```python
from build123d import *

# Parameters (mm, degrees)
EXTRUDE_1_DEPTH     = 7
FILLET_1_R          = 5
CUT_EXTRUDE_1_REACH = 193.047
SKETCH_3_R          = 3.5


with BuildPart() as part:
    # 草图1 → 凸台-拉伸1 (new, symmetric)
    with BuildSketch(Plane.XY):
        Polygon((0, 150), (-15, 150), (-15, 15), (-135, 15), (-135, 0), (0, 0), align=None)
    extrude(amount=EXTRUDE_1_DEPTH, both=True)

    # 圆角1
    fillet_1_edges = [part.edges().sort_by_distance(p)[0] for p in [
        (-15, 15, 0),
    ]]
    fillet(fillet_1_edges, radius=FILLET_1_R)

    # 草图3 → 切除-拉伸1 (cut, up to next)
    with BuildSketch(Plane(origin=(0, 15, 0), x_dir=(1, 0, 0), z_dir=(0, 1, 0)), mode=Mode.PRIVATE) as cut_extrude_1_sk1:
        with Locations(Location((-127, 0, 0), (0, 0, 180))):
            Circle(SKETCH_3_R)
    cut_extrude_1_tool1 = extrude(cut_extrude_1_sk1.sketch, amount=-CUT_EXTRUDE_1_REACH, mode=Mode.PRIVATE) & part.part
    # 草图3 → 切除-拉伸1 (cut, up to next)
    with BuildSketch(Plane(origin=(0, 15, 0), x_dir=(1, 0, 0), z_dir=(0, 1, 0)), mode=Mode.PRIVATE) as cut_extrude_1_sk2:
        with Locations(Location((-105, 0, 0), (0, 0, 180))):
            Circle(SKETCH_3_R)
    cut_extrude_1_tool2 = extrude(cut_extrude_1_sk2.sketch, amount=-CUT_EXTRUDE_1_REACH, mode=Mode.PRIVATE) & part.part
    add(cut_extrude_1_tool1.solids().sort_by_distance((-127, 15, 0))[0], mode=Mode.SUBTRACT)
    add(cut_extrude_1_tool2.solids().sort_by_distance((-105, 15, 0))[0], mode=Mode.SUBTRACT)


solid = part.part
```
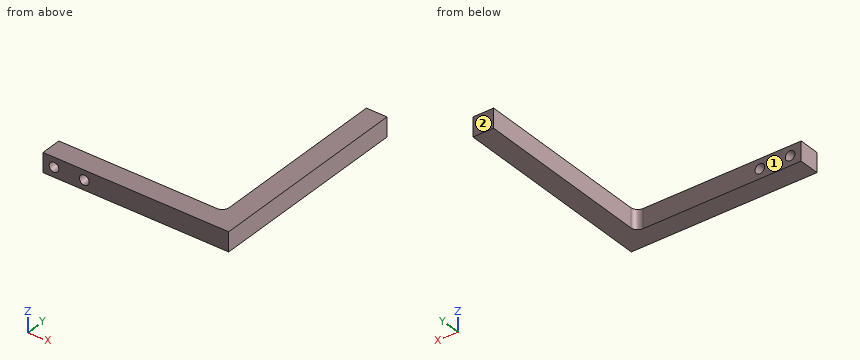
Design review of the part built by this model. Coordinates are the model's own, in mm. Face numbers are marked on the shaded views. A direction names the side the tool comes from. Give positions to 0.01 mm unless a question says otherwise; leave off trailing zeros. Order: outer loops, then holes, each group sorted by start corner. A loop starts at its lowest first (then second) coordinate and runs counter-clockwise, first axis right, second up. Notation, with made-up numbers: (88.25, 21) -> (105.25, 21) arc R29 cw to (105.25, 49) -> close; hole circle Ø4 at (3.5, 12.25). An arc over 180 degrees is marked (long way). Write item = value, one per line. Start each with the question number.
(1) For pin 1 (8 mm diameter, centred on x = -21.5, z = 2, fed in from +Y); pin 2 (5 mm diameter, centred on x = -65.5, z = 1.5, fed in from -Y); pin 3 (6.5 mm diameter, centred on x = -105, z = 0, fed in from -Y); pin 4 (4 mm diameter, centred on x = -86, z = -2, fed in from +Y), all flat-tipped, find the tip position at first contact; note any pin that passes through.
(2) For the marked faces 1 and 2, list the 3-axis set-ups (+Z, -Z, +X, -X, +Y, -Y) from which the entire face can be reached by the end or side of a thin tool; tool diameter is ignored.
(3) We need section D-D on y = 107. Write out the cut boundary in (x, z), plus the area to 3 significant figures.
(4) To check wall thickness, follow line 1 along Z through (x, y) = (-105, 10.5); line 2 along Y through (x, z) = (-120.5, -2.25); line 3 along X through (y, z) = (108, -5). State the ranges of each line that lie inside material, in increasing order.
(5) We need section A-A on z = 0. Write out the cut boundary in (x, y), plus the area to 3 significant figures.
(6) We need section C-C on x = -126.5. Write out the cut boundary in (y, z).
(7) We need section B-B on x = -105. Write out the cut boundary in (y, z), plus the area to 3 significant figures.
Numbers:
q1.pin_1 = 15.67
q1.pin_2 = 0
q1.pin_3 = through
q1.pin_4 = 15
q2.face_1 = +Z, -Z, -X, +Y
q2.face_2 = +Z, -Z, +X, -X, +Y
q3.outline = (-15, -7) -> (0, -7) -> (0, 7) -> (-15, 7) -> close
q3.area = 210 mm^2
q4.line_1 = -7 to -3.5, 3.5 to 7
q4.line_2 = 0 to 15
q4.line_3 = -15 to 0
q5.outline = (-135, 0) -> (-130.5, 0) -> (-130.5, 15) -> (-135, 15) -> close; (-123.5, 0) -> (-108.5, 0) -> (-108.5, 15) -> (-123.5, 15) -> close; (-101.5, 0) -> (0, 0) -> (0, 150) -> (-15, 150) -> (-15, 20) arc R5 cw to (-20, 15) -> (-101.5, 15) -> close
q5.area = 3,850 mm^2
q6.outline = (0, -7) -> (15, -7) -> (15, -3.46) -> (0, -3.46) -> close; (0, 3.46) -> (15, 3.46) -> (15, 7) -> (0, 7) -> close
q7.outline = (0, -7) -> (15, -7) -> (15, -3.5) -> (0, -3.5) -> close; (0, 3.5) -> (15, 3.5) -> (15, 7) -> (0, 7) -> close
q7.area = 105 mm^2
